Job drawing, mm, ordinate dimensions from the low corner. One solid piece. A direction names the side the tool comes from. Round coordinates to 2 decimals unless told otherwise and drop trailing zeros. Order: outer loops, then holes, each group sorted by start corner. A loop starts at its lowest first (then second) coordinate and runs counter-clockwise, first axis right, second up. Notation, with made-up numbers: (38.5, 67.25) - (87.5, 67.25) arc R21 cw to (87.5, 76.25) - close; hole circle Ø1 at (22.5, 59). An arc over 180 degrees is marked (long way). Write each question's results on one line, items separated by ' | '. Start each with the question number.
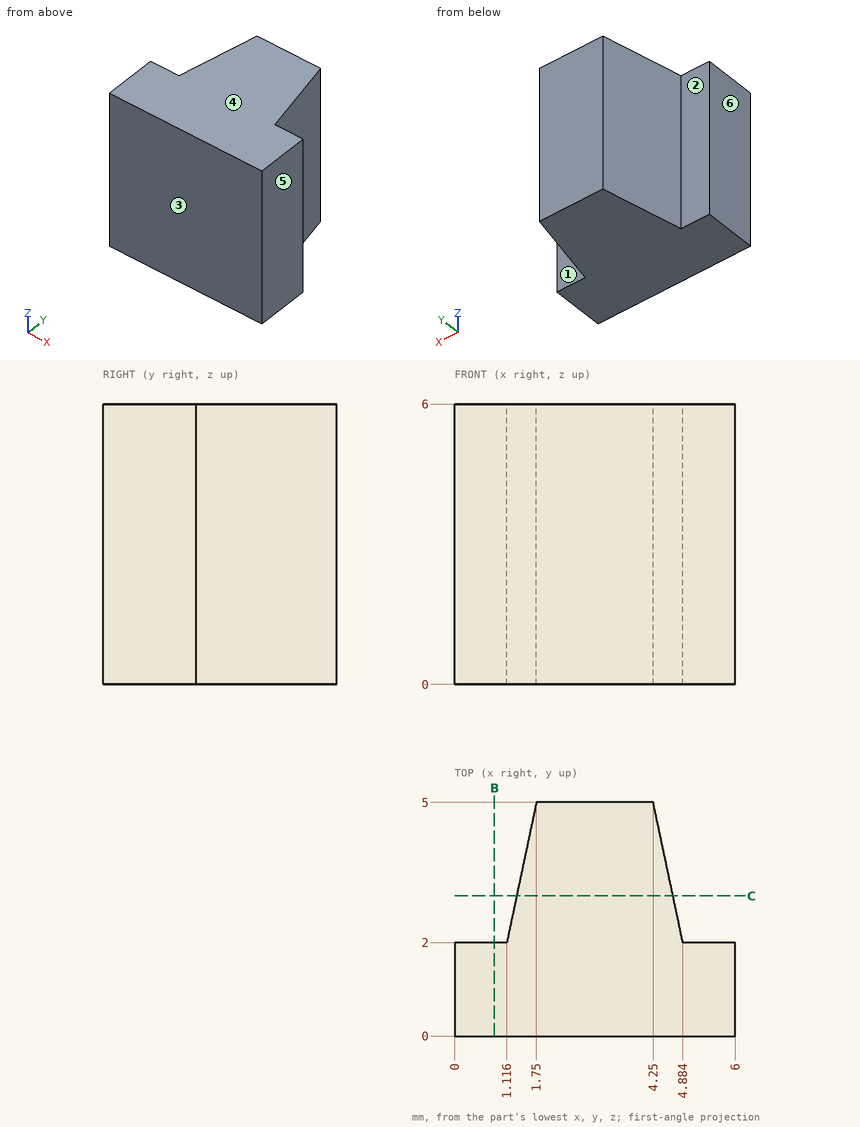
1. Mould opens along X. For the marked faces 4, 5 and 6 say: pulls with the +X half, pulls with the -X half, needs draft (parallel to the pull), parting line crosses it, or undercut.
2. 3-axis set-ups, long thin cutter, end or side, ignore diameter. For the marked faces 1, 2 and 3: which of +Z, -Z, +X, -X, +Y, -Y reach the whole face in a straight line?
3. Cut at B-B (x = 0.85). List the corners of the cut face in (y, z).
4. Flat gauge pins, fed straight in: pin 1 Ø0.9 at (x, z) = (0.5, 3.5) entering from +Y; pin 2 Ø3 at (y, z) = (1.5, 5) entering from -X. Where does each tip first touch, or does it go through?
5. Wall check: line 1 (Y direction, x = 5.65, z = 3.1); line 2 (X direction, y = 3.75, z = 2.85) (1 decimal); line 3 (X direction, y = 2.5, z = 3.9). Give the ranges that are in metal, low to high. Write a range as from..to.
6. Cut at C-C (y = 3). List the corners of the cut face in (x, z), plus the area to 3 significant figures.
A:
1) face 4: needs draft | face 5: pulls with the +X half | face 6: pulls with the -X half
2) face 1: +Z, -Z, +X, +Y | face 2: +Z, -Z, -X, +Y | face 3: +Z, -Z, +X, -X, -Y
3) outline: (0, 0) - (2, 0) - (2, 6) - (0, 6) - close
4) pin 1: stops at y = 2 | pin 2: stops at x = 0
5) line 1: y = 0..2 | line 2: x = 1.5..4.5 | line 3: x = 1.22..4.78
6) outline: (1.33, 0) - (4.67, 0) - (4.67, 6) - (1.33, 6) - close | area: 20.1 mm^2
